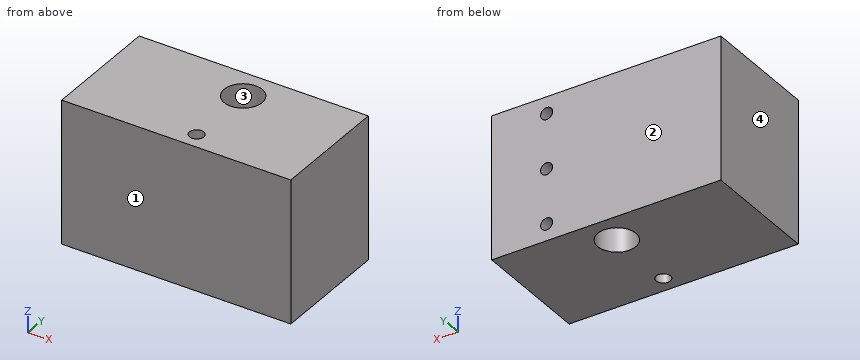
from build123d import *

# Parameters (mm, degrees)
SKETCH1_W             = 48
SKETCH1_H             = 30
BOSS_EXTRUDE1_DEPTH   = 25
CUT_EXTRUDE2_REACH    = 47.837
SKETCH3_R             = 4
SKETCH3_R_2           = 1.5
SKETCH4_R             = 1
CUT_EXTRUDE3_DEPTH    = 2
M3_TAPPED_HOLE1_D     = 2.5
M3_TAPPED_HOLE1_DEPTH = 7.5
M3_TAPPED_HOLE1_TIP   = 0.751075774


with BuildPart() as part:
    # Sketch1 → Boss-Extrude1 (new body)
    with BuildSketch(Plane(origin=(0, 0, 0), x_dir=(1, 0, 0), z_dir=(0, 1, 0))):
        Rectangle(SKETCH1_W, SKETCH1_H)
    extrude(amount=BOSS_EXTRUDE1_DEPTH)

    # Sketch3 → Cut-Extrude2 (cut, up to next)
    with BuildSketch(Plane.XY.offset(15), mode=Mode.PRIVATE) as cut_extrude2_sk1:
        with Locations((2, 18.5)):
            Circle(SKETCH3_R)
    cut_extrude2_tool1 = extrude(cut_extrude2_sk1.sketch, amount=-CUT_EXTRUDE2_REACH, mode=Mode.PRIVATE) & part.part
    # Sketch3 → Cut-Extrude2 (cut, up to next)
    with BuildSketch(Plane.XY.offset(15), mode=Mode.PRIVATE) as cut_extrude2_sk2:
        with Locations((2, 3.5)):
            Circle(SKETCH3_R_2)
    cut_extrude2_tool2 = extrude(cut_extrude2_sk2.sketch, amount=-CUT_EXTRUDE2_REACH, mode=Mode.PRIVATE) & part.part
    add(cut_extrude2_tool1.solids().sort_by_distance((2, 18.5, 15))[0], mode=Mode.SUBTRACT)
    add(cut_extrude2_tool2.solids().sort_by_distance((2, 3.5, 15))[0], mode=Mode.SUBTRACT)

    # Sketch4 → Cut-Extrude3 (cut)
    with BuildSketch(Plane(origin=(0, 25, 0), x_dir=(1, 0, 0), z_dir=(0, 1, 0))):
        with Locations(Location((12.5, 11.5, 0), (0, 0, 270))):
            Circle(SKETCH4_R)
        with Locations(Location((12.5, 0, 0), (0, 0, 270))):
            Circle(SKETCH4_R)
        with Locations(Location((12.5, -11.5, 0), (0, 0, 270))):
            Circle(SKETCH4_R)
    extrude(amount=-CUT_EXTRUDE3_DEPTH, mode=Mode.SUBTRACT)

    # M3 Tapped Hole1
    with Locations(Plane(origin=(0, 25, 0), x_dir=(1, 0, 0), z_dir=(0, 1, 0))):
        with Locations((12.5, 11.5), (12.5, 0), (12.5, -11.5)):
            Hole(M3_TAPPED_HOLE1_D / 2, depth=M3_TAPPED_HOLE1_DEPTH)
            with Locations((0, 0, -(M3_TAPPED_HOLE1_DEPTH + M3_TAPPED_HOLE1_TIP / 2))):  # 118° drill point
                Cone(0, M3_TAPPED_HOLE1_D / 2, M3_TAPPED_HOLE1_TIP, mode=Mode.SUBTRACT)


solid = part.part
Input: part model. Units: mm. Frame: model coordinates. Face numbers are marked on the shaded views. Round coordinates to 2 decimals unless told otherwise and drop trailing zeros. Order: outer loops, then holes, each group sorted by start corner. A loop starts at its lowest first (then second) coordinate and runs counter-clockwise, first axis right, second up. Notation, with made-up numbers: (41, 8) - (61, 8) arc R13 cw to (61, 18) - close; hole circle Ø4 at (67.5, -18). An arc over 180 degrees is marked (long way). Answer as a JSON object with one key per item and string values. Group by question number.
(1) Cut plane A-A (y = 18.5). Return loops of the section in (x, z).
(2) Cut plane B-B (z = -8). Return loops of the section in (x, y), then the cut area to 3 significant figures.
(3) Material intervals for probe 1 along Z at (x, y) = (12.5, 22.5); probe 2 along Y at (x, z) = (2, -4.5); probe 3 along X at (y, z) = (23.25, 11.5), sorted ascending. Write a range as from..to.
(4) Draft query along Y for the marked faces 1, 2, 3 and 4. Return one class per face: released by +Y, released by -Y, zero draft, split by the parting line, or undercut.
(5) Pin query (flat end, axial travel): P1, Ø2, axis at x = 12.5, z = 11.5, coming from the +Y side. Return the tip coordinate at first contact, or that it passes through.
(6) Cut plane C-C (x = 2). Return loops of the section in (y, z), then the cut area to 3 significant figures.
Here are the results:
{
 "1": {"outline": "(-24, -15) - (-2, -15) - (-2, 15) - (-24, 15) - close; (6, -15) - (24, -15) - (24, 15) - (6, 15) - close; hole circle Ø2.5 at (12.5, -11.5); hole circle Ø2.5 at (12.5, 0); hole circle Ø2.5 at (12.5, 11.5)"},
 "2": {"outline": "(-24, 0) - (24, 0) - (24, 25) - (-24, 25) - close; hole circle Ø8 at (2, 18.5); hole circle Ø3 at (2, 3.5)", "area": "1,140 mm^2"},
 "3": {"probe 1": "z = -15..-12.75, -10.25..-1.25, 1.25..10.25, 12.75..15", "probe 2": "y = 0..2, 5..14.5, 22.5..25", "probe 3": "x = -24..11.25, 13.75..24"},
 "4": {"face 1": "released by -Y", "face 2": "released by +Y", "face 3": "undercut", "face 4": "zero draft"},
 "5": {"P1": "stops at y = 17.35"},
 "6": {"outline": "(0, -15) - (2, -15) - (2, 15) - (0, 15) - close; (5, -15) - (14.5, -15) - (14.5, 15) - (5, 15) - close; (22.5, -15) - (25, -15) - (25, 15) - (22.5, 15) - close", "area": "420 mm^2"}
}
